Here's the drawing with two shaded views (mm, measured from the low corner). I have some questions. Round coordinates to 2 decimals unless told otherwise and drop trailing zeros. Loops run counter-clockwise (first coordinate to the right, second up) from the corner with the lowest first, then second, coordinate; pieces in that order, holes last. Notation, with made-up numbers: (2, 35.5) -> (8, 35.5) arc R17 ccw to (8, 42.5) -> close; hole circle Ø8 at (76, 53.5). An arc over 180 degrees is marked (long way). Use a Markdown table: item, result.
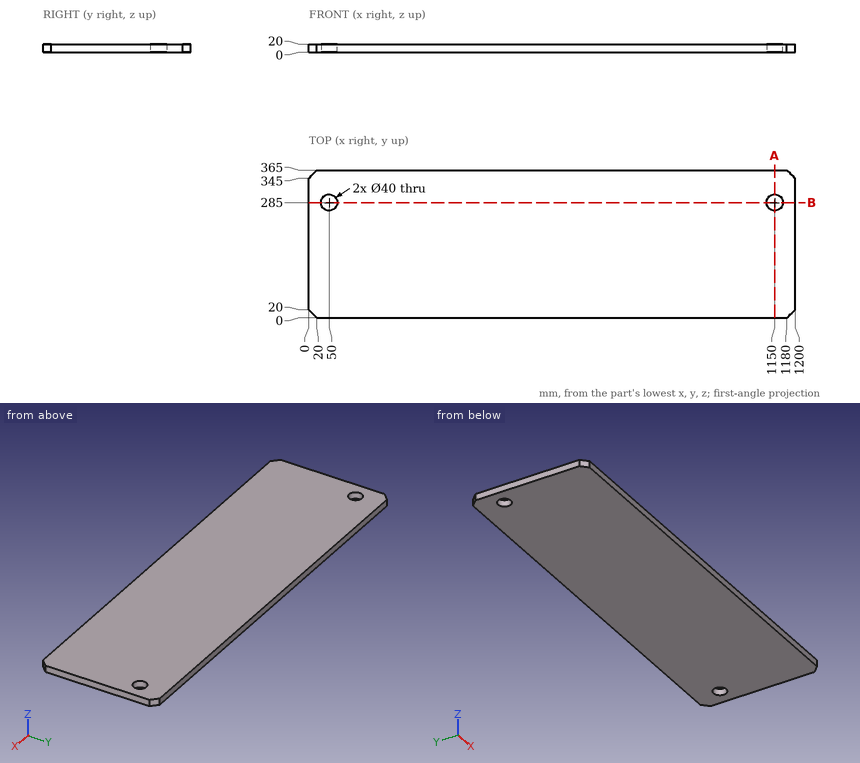
1. I want a section at B-B (y = 285). Please give me the cut outline in (x, z).
Answer sheet:
| item | result |
|---|---|
| outline | (0, 0) -> (30, 0) -> (30, 20) -> (0, 20) -> close; (70, 0) -> (1130, 0) -> (1130, 20) -> (70, 20) -> close; (1170, 0) -> (1200, 0) -> (1200, 20) -> (1170, 20) -> close |
2. I need wall thicknesses on line 1 (X direction, y = 285, z = 12); line 2 (Y direction, x = 1150, z = 11.75); line 3 (X direction, y = 273.5, z = 5.25). Which ranges of each line are inside material? Lowest first, please.
Answer sheet:
| item | result |
|---|---|
| line 1 | x = 0 to 30, 70 to 1130, 1170 to 1200 |
| line 2 | y = 0 to 265, 305 to 365 |
| line 3 | x = 0 to 33.64, 66.36 to 1133.64, 1166.36 to 1200 |
3. I want a section at A-A (x = 1150). Please give me the cut outline in (y, z), plus the area to 3 significant figures.
Answer sheet:
| item | result |
|---|---|
| outline | (0, 0) -> (265, 0) -> (265, 20) -> (0, 20) -> close; (305, 0) -> (365, 0) -> (365, 20) -> (305, 20) -> close |
| area | 6,500 mm² |
